Geometry: see drawing. Coordinates: mm, zero at the bounding-box minimum. A direction names the side the tool comes from. Give positions to 0.01 mm unless a question says otherwise; leave off trailing zeros. Write each loop counter-clockwise with the first axis right and the second up, starting at its lowest first coordinate (ties: lowest second). Pieces come first, ordered by that corner, then holes. Notation, with made-up numbers: (32.25, 59.5) - (63.25, 59.5) arc R20 ccw to (63.25, 81.5) - close; hole circle Ø10 at (63.5, 28). An arc over 180 degrees is marked (long way). Return JSON: item names as keys, results as strings.
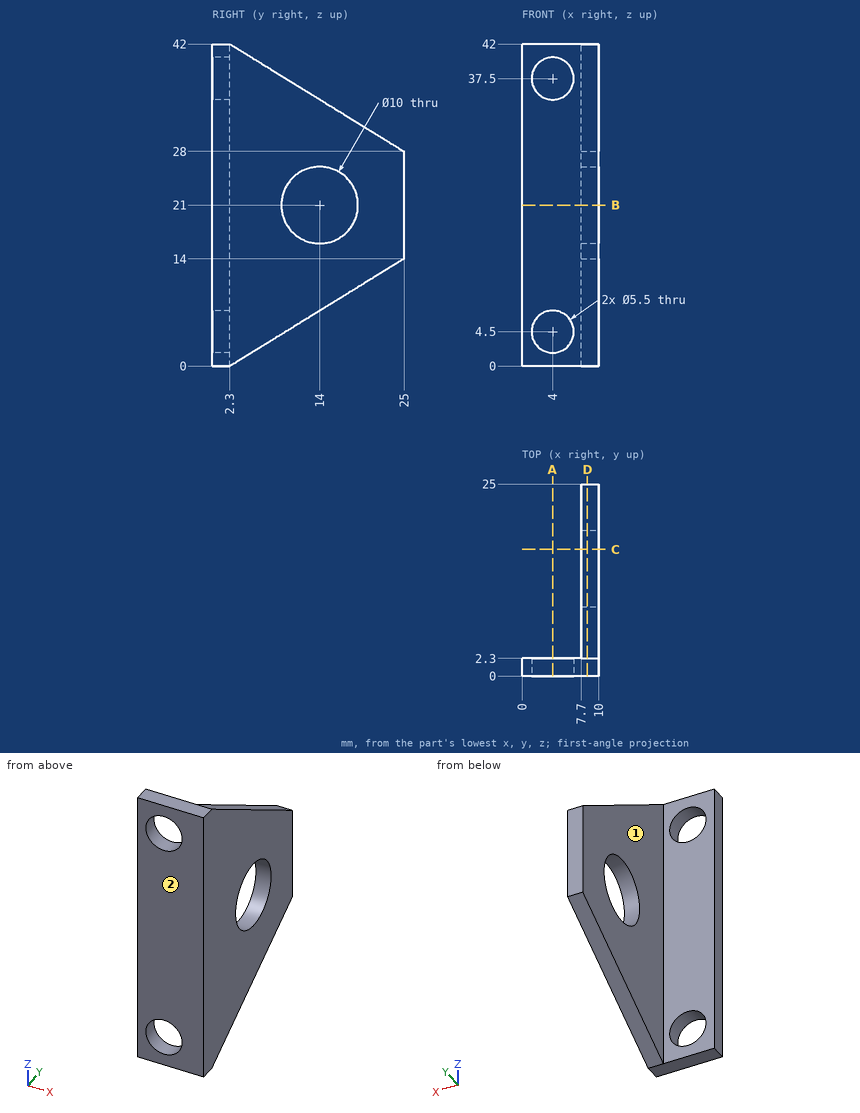
Q1. Set-up query: the marked faces 1 and 2. Return all of +Z, -Z, +X, -X, +Y, -Y with unobstructed straight access to the full face (end or side cutting, diameter ignored); none if empty.
Answer key:
{"face 1": "+Z, -Z, -X, +Y", "face 2": "+Z, -Z, +X, -X, -Y"}
Q2. Pin query (flat end, axial travel): P1, Ø3, axis at x = 7, y = 8, coming from the +Z side; P2, Ø4.5, axis at x = 4, z = 4.5, coming from the +Y side; P3, Ø10, axis at y = 17.5, z = 15, coming from the -X side; P4, Ø2.5, axis at x = 5.5, z = 10.5, coming from the +Y side. Return the tip coordinate at first contact, or that it passes through.
Answer key:
{"P1": "stops at z = 39.3", "P2": "passes through", "P3": "stops at x = 7.7", "P4": "stops at y = 2.3"}
Q3. Section query D-D, the plane x = 8.5. Return the cut outline in (y, z).
Answer key:
{"outline": "(0, 0) - (2.3, 0) - (25, 14) - (25, 28) - (2.3, 42) - (0, 42) - close; hole circle Ø10 at (14, 21)"}
Q4. Material intervals for probe 1 along Z at (x, y) = (4, 1.35); probe 2 along X at (y, z) = (4.5, 2.5); probe 3 along Y at (x, z) = (5.25, 21), sorted ascending. Write a range as [from, to].
Answer key:
{"probe 1": "z = [0, 1.75], [7.25, 34.75], [40.25, 42]", "probe 2": "x = [7.7, 10]", "probe 3": "y = [0, 2.3]"}
Q5. Section query C-C, the plane y = 16.5. Return the cut outline in (x, z), plus the area to 3 significant figures.
Answer key:
{"outline": "(7.7, 8.76) - (10, 8.76) - (10, 16.67) - (7.7, 16.67) - close; (7.7, 25.33) - (10, 25.33) - (10, 33.24) - (7.7, 33.24) - close", "area": "36.4 mm^2"}
Q6. Section query B-B, the plane z = 21. Return the cut outline in (x, y), plus the area to 3 significant figures.
Answer key:
{"outline": "(0, 0) - (10, 0) - (10, 9) - (7.7, 9) - (7.7, 2.3) - (0, 2.3) - close; (7.7, 19) - (10, 19) - (10, 25) - (7.7, 25) - close", "area": "52.2 mm^2"}
Q7. Section query A-A, the plane x = 4. Return the cut outline in (y, z).
Answer key:
{"outline": "(0, 0) - (2.3, 0) - (2.3, 1.75) - (0, 1.75) - close; (0, 7.25) - (2.3, 7.25) - (2.3, 34.75) - (0, 34.75) - close; (0, 40.25) - (2.3, 40.25) - (2.3, 42) - (0, 42) - close"}
